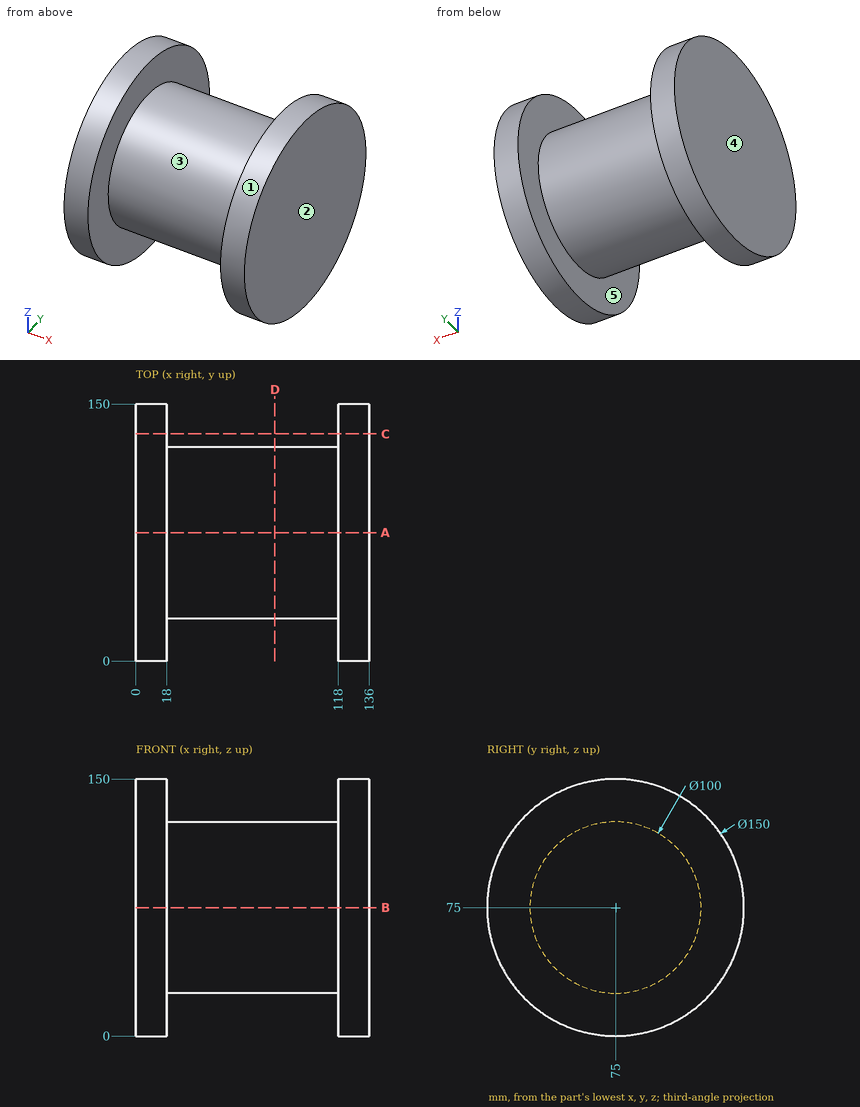
Study the drawing (mm; zero at the part's minimum x, y, z) and answer. A direction names the side the tool comes from. Give positions to 0.01 mm unless a question says otherwise; leave off trailing zeros. Write each loop counter-clockwise with the first axis right and the second up, starting at its lowest first coordinate (ties: lowest second). Pieces come first, ordered by that corner, then holes.
Item 1: Which of the six approach directions +Z, -Z, +X, -X, +Y, -Y give full straight-line access (tool end or side, diameter ignored) to the marked faces 4 and 5?
Item 2: Section A-A, the plane y = 75 is taken. Write down the section's boundary in (x, z).
Item 3: Flat-ended cylindrical pins translate along their axes: P1, Ø8, axis at x = 101.5, z = 33.5, coming from the -Y side; P2, Ø4, axis at x = 18, z = 64.5, coming from the -Y side; P3, Ø2, axis at x = 102, z = 54, coming from the +Y side. Find the tip coordinate at first contact, or state that the pin passes through.
Item 4: Find the intervals of material crossed by line 1 along X through (y, z) = (79, 20.5); line 2 along Z through (x, y) = (81.5, 72); line 3 along Z through (x, y) = (52.5, 37), in increasing order.
Item 5: Determine the mould class of the marked faces 1, 2 and 3 for opening direction X: released by +X, released by -X, zero draft, split by the parting line, or undercut.
Item 6: Section D-D, the plane x = 81 is taken. Write down the section's boundary in (y, z).
Item 7: Section C-C, the plane y = 132.5 is taken. Write down the section's boundary in (x, z), plus the area to 3 significant figures.
Completed:
1. face 4: +Z, -Z, -X, +Y, -Y
1. face 5: none
2. outline: (0, 0) - (18, 0) - (18, 25) - (118, 25) - (118, 0) - (136, 0) - (136, 150) - (118, 150) - (118, 125) - (18, 125) - (18, 150) - (0, 150) - close
3. P1: stops at y = 41.93
3. P2: stops at y = 0.48
3. P3: stops at y = 120.83
4. line 1: x = 0 to 18, 118 to 136
4. line 2: z = 25.09 to 124.91
4. line 3: z = 42.5 to 107.5
5. face 1: zero draft
5. face 2: released by +X
5. face 3: undercut
6. outline: circle Ø100 at (75, 75)
7. outline: (0, 26.85) - (18, 26.85) - (18, 123.15) - (0, 123.15) - close; (118, 26.85) - (136, 26.85) - (136, 123.15) - (118, 123.15) - close
7. area: 3,470 mm2
